The figure shows three views and two pictorial views of one solid part (mm, origin at its lowest corner). Answer the questions. A direction names the side the tool comes from. Give positions to 0.01 mm unless a question says otherwise; leave off trailing zeros. Write each loop counter-clockwise with the first axis right and the second up, starting at its lowest first coordinate (ties: lowest second). Pieces come first, ordered by that corner, then holes. Notation, with made-up numbers: (44.25, -1) -> (48.25, -1) arc R25 cw to (48.25, 17) -> close; hole circle Ø1 at (59.25, 45.5). An arc over 180 degrees is marked (long way). Write each question's results on one line, items separated by ' | '. Start each with the question number.
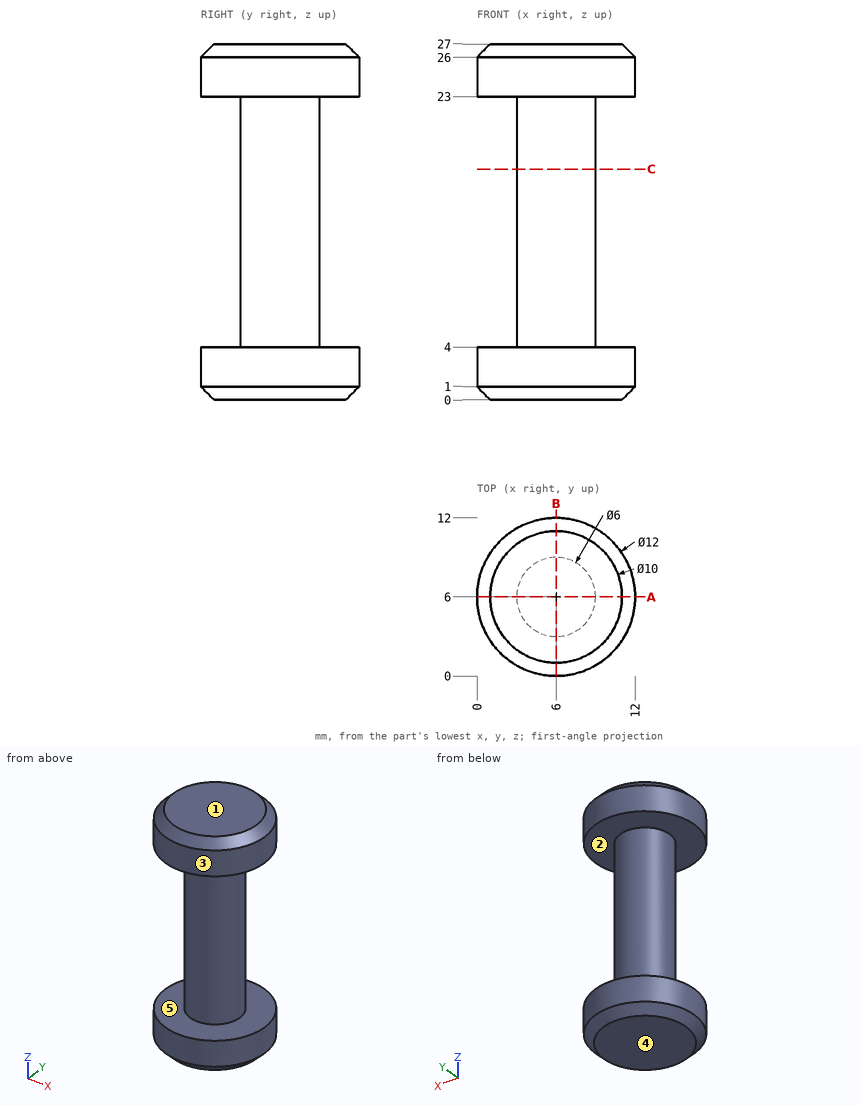
1. A tool of negligible diameter and unlimited length cuts with its end or side. For the marked faces 1 and 2, from which of +Z, -Z, +X, -X, +Y, -Y can it reach the whole face along a straight path? Write none if from no direction.
2. Each of these flat-tipped pins is pushed along its axis until it touches: pin 1 Ø1.5 at (x, z) = (6, 12.5) entering from +Y; pin 2 Ø5 at (x, z) = (5.5, 13) entering from -Y; pin 3 Ø1.5 at (y, z) = (8.5, 14.5) entering from -X. Where does it stop, or does it pass through?
3. Section A-A (y = 6) is taken. Write down the section's boundary in (x, z).
4. The mould has two halves that part along Z. Classify the marked faces 3, 4 and 5: pulls with the +Z half, pulls with the -Z half, needs draft (parallel to the pull), parting line crosses it, or undercut.
5. Consider probe 1 along Z at (x, y) = (2.25, 7.25); probe 2 along Z at (x, y) = (2.25, 1.75); probe 3 along X at (y, z) = (5.75, 19.5). Determine where each line is inside the solid, lowest interval first. Write a range as [from, to].
6. Section C-C (z = 17.5) is taken. Write down the section's boundary in (x, y).
Results:
1) face 1: +Z, +X, -X, +Y, -Y | face 2: none
2) pin 1: stops at y = 9 | pin 2: stops at y = 3 | pin 3: stops at x = 3.56
3) outline: (0, 1) -> (1, 0) -> (11, 0) -> (12, 1) -> (12, 4) -> (9, 4) -> (9, 23) -> (12, 23) -> (12, 26) -> (11, 27) -> (1, 27) -> (0, 26) -> (0, 23) -> (3, 23) -> (3, 4) -> (0, 4) -> close
4) face 3: needs draft | face 4: pulls with the -Z half | face 5: undercut
5) probe 1: z = [0, 4], [23, 27] | probe 2: z = [0.67, 4], [23, 26.33] | probe 3: x = [3.01, 8.99]
6) outline: circle Ø6 at (6, 6)
